Geometry check sheet. Reference: drawing and pictorial views, mm from the part's lowest x, y, z. Give positions to 0.01 mm unless a question says otherwise; leave off trailing zeros. Order: outer loops, then holes, each group sorted by start corner. A loop starts at its lowest first (then second) coordinate and runs counter-clockwise, first axis right, second up. Notation, with made-up numbers: (-25, 73) - (19, 73) arc R20 ccw to (19, 101) - close; hole circle Ø8 at (68.5, 84). An arc over 180 degrees is marked (long way). Answer in a Markdown table with one row per item.
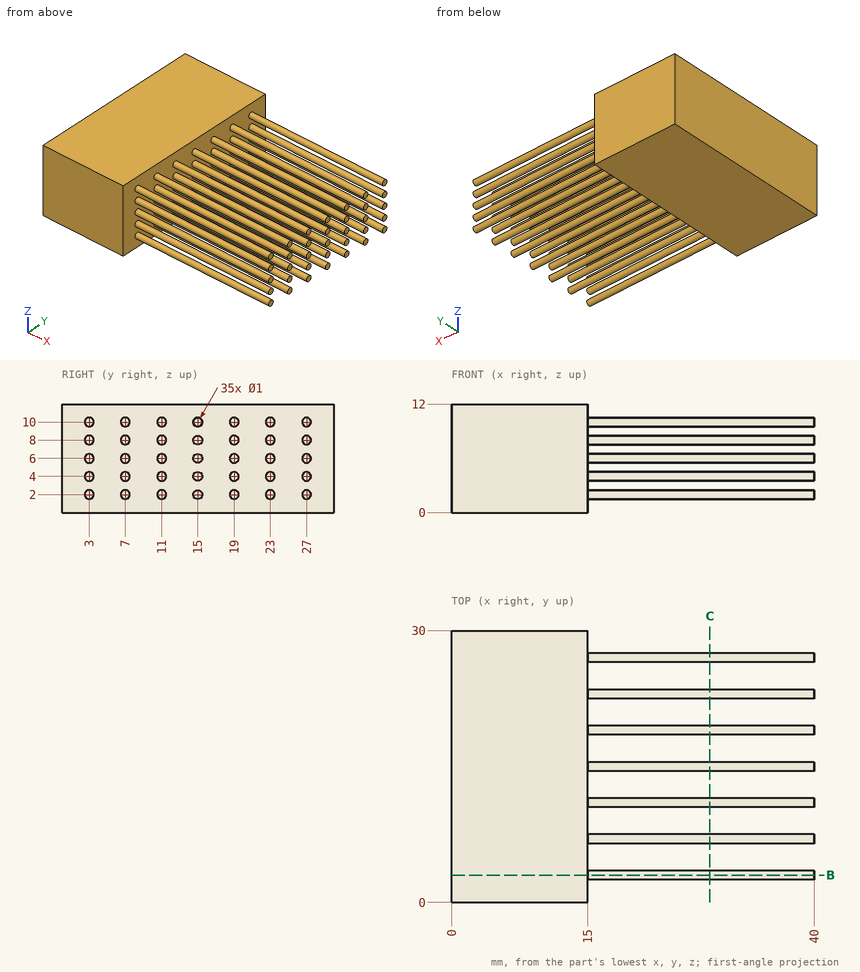
(1) Cross-section at B-B, the plane y = 3. Record the cut outline in (x, z), then the cut area to 3 significant figures.
Geometry says:
| item | result |
|---|---|
| outline | (0, 0) - (15, 0) - (15, 1.5) - (40, 1.5) - (40, 2.5) - (15, 2.5) - (15, 3.5) - (40, 3.5) - (40, 4.5) - (15, 4.5) - (15, 5.5) - (40, 5.5) - (40, 6.5) - (15, 6.5) - (15, 7.5) - (40, 7.5) - (40, 8.5) - (15, 8.5) - (15, 9.5) - (40, 9.5) - (40, 10.5) - (15, 10.5) - (15, 12) - (0, 12) - close |
| area | 305 mm² |
(2) Cross-section at C-C, the plane x = 28.5. Give the number of separate pieces and of enclosed holes in the cut face, then the cut area to 3 significant figures.
Geometry says:
| item | result |
|---|---|
| separate pieces | 35 |
| enclosed holes | 0 |
| area | 27.5 mm² |
(3) Thickness scan on L1, parallel to Z at x = 23, y = 23; L2, parallel to X at y = 18.25, z = 8.5. Record the ranges inside material, lowest first.
Geometry says:
| item | result |
|---|---|
| L1 | 1.5 to 2.5, 3.5 to 4.5, 5.5 to 6.5, 7.5 to 8.5, 9.5 to 10.5 |
| L2 | 0 to 15 |
(4) Gauge pin test, flat ends, axial feed: P1, Ø5, axis at x = 24.5, y = 23.5, coming from the +Z side; P2, Ø6, axis at x = 27.5, z = 3, coming from the +Y side; P3, Ø2, axis at x = 16.5, z = 5, coming from the -Y side. Record the tip position at first contact, or that the pin passes through.
Geometry says:
| item | result |
|---|---|
| P1 | z = 10.5 |
| P2 | y = 27.5 |
| P3 | y = 2.5 |
